from build123d import *

# Parameters (mm, degrees)
SKETCH1_R           = 4
BOSS_EXTRUDE1_DEPTH = 10


with BuildPart() as part:
    # Sketch1 → Boss-Extrude1 (new body)
    with BuildSketch(Plane.XY):
        with BuildLine():
            Line((0, 7.5), (100, 7.5))
            ThreePointArc((100, 7.5), (107.5, 0), (100, -7.5))
            Line((100, -7.5), (0, -7.5))
            ThreePointArc((0, -7.5), (-7.5, 0), (0, 7.5))
        make_face()
        Circle(SKETCH1_R, mode=Mode.SUBTRACT)
        with Locations((100, 0)):
            Circle(SKETCH1_R, mode=Mode.SUBTRACT)
    extrude(amount=BOSS_EXTRUDE1_DEPTH)


solid = part.part
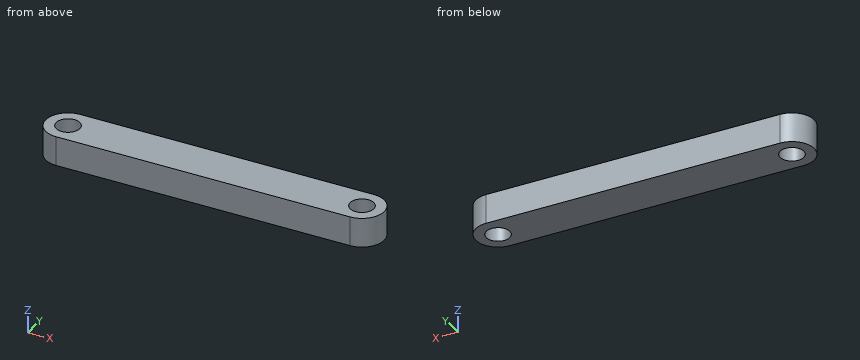
Build history of the part. All positions in model axes, mm. Coordinates: 2 decimals unless noted, no trailing zeros. Order: outer loops, then holes, each group sorted by start corner. A loop starts at its lowest first (then second) coordinate and runs counter-clockwise, first axis right, second up. Notation, with made-up numbers: (42, 70) - (69, 70) arc R29 ccw to (69, 108) - close; hole circle Ø11 at (66.5, -15.5). An arc over 180 degrees is marked (long way). Write item = value, one per line. Start each with the question number.
1) Saw through at A-A on y = 0. Write the cut outline in (x, z).
2) Saw through at C-C on y = 6.5. Write the cut outline in (x, z).
3) Flat gauge pins, fed straight in: pin 1 Ø5 at (y, z) = (4.5, 5) entering from +X; pin 2 Ø2 at (y, z) = (-2.5, 1) entering from -X. Where does each tip first touch, or does it go through?
4) Saw through at B-B on z = 7.25. Write the cut outline in (x, y), then the cut area to 3 significant figures.
5) Saw through at D-D on y = -5.25. Write the cut outline in (x, z).
6) Wall check: line 1 along Y through (x, z) = (100, 7.25); line 2 along X through (y, z) = (-1.25, 0.5); line 3 along X through (y, z) = (-1.5, 4.25). Give the ranges that are in metal, low to high. Write a range as from..to.
From the geometry:
q1.outline = (-7.5, 0) - (-4, 0) - (-4, 10) - (-7.5, 10) - close; (4, 0) - (96, 0) - (96, 10) - (4, 10) - close; (104, 0) - (107.5, 0) - (107.5, 10) - (104, 10) - close
q2.outline = (-3.74, 0) - (103.74, 0) - (103.74, 10) - (-3.74, 10) - close
q3.pin_1 = 107.23
q3.pin_2 = -7.35
q4.outline = (0, -7.5) - (100, -7.5) arc R7.5 ccw to (100, 7.5) - (0, 7.5) arc R7.5 ccw to start; hole circle Ø8 at (0, 0); hole circle Ø8 at (100, 0)
q4.area = 1,580 mm^2
q5.outline = (-5.36, 0) - (105.36, 0) - (105.36, 10) - (-5.36, 10) - close
q6.line_1 = -7.5..-4, 4..7.5
q6.line_2 = -7.4..-3.8, 3.8..96.2, 103.8..107.4
q6.line_3 = -7.35..-3.71, 3.71..96.29, 103.71..107.35
